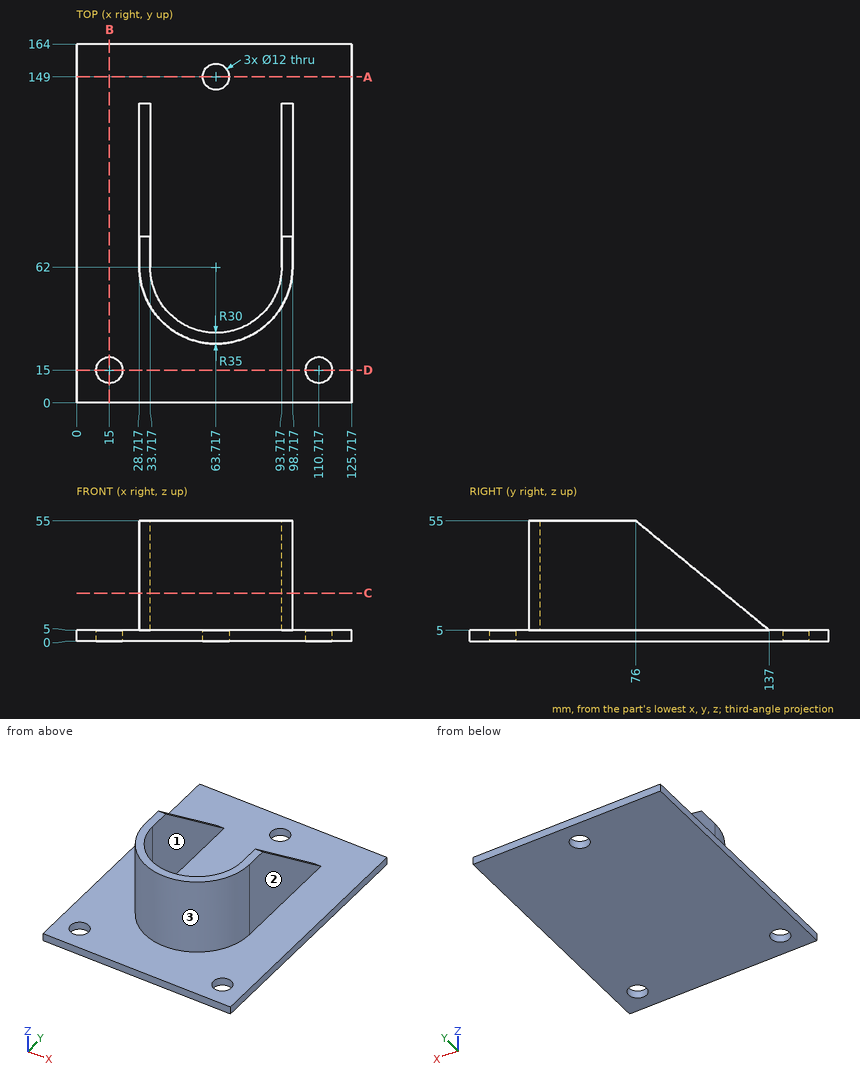
Input: dimensioned drawing with shaded views. Units: mm. Origin: part minimum x, y, z. Round coordinates to 2 decimals unless told otherwise and drop trailing zeros. Order: outer loops, then holes, each group sorted by start corner. A loop starts at its lowest first (then second) coordinate and runs counter-clockwise, first axis right, second up. Notation, with made-up numbers: (-23.75, 67) -> (13.25, 67) arc R24 ccw to (13.25, 84) -> close; hole circle Ø7 at (82, -20.5). An arc over 180 degrees is marked (long way). One line per item, written item: value. Start each with the question number.
Q1. Section query C-C (z = 22). Return the cut outline in (x, y), plus the area to 3 significant figures.
Q2. Section query D-D (y = 15). Return the cut outline in (x, z).
Q3. Section query B-B (x = 15). Return the cut outline in (y, z).
Q4. Draft query along X for the marked faces 1, 2 and 3. Return one class per face: pulls with the +X half, pulls with the -X half, needs draft (parallel to the pull), parting line crosses it, or undercut.
Q5. Section query A-A (y = 149). Return the cut outline in (x, z).
Q6. Pin query (flat end, axial travel): pin 1 (25 mm diameter, centred on y = 105, z = 39.5, fed in from -X); pin 2 (10 mm diameter, centred on y = 45, z = 11.5, fed in from +X); pin 3 (5 mm diameter, centred on y = 91.5, z = 32.5, fed in from +X). Return the tip coordinate at first contact, or that it passes through.
Q7. Material intervals for probe 1 along X at (y, z) = (72, 43); probe 2 along Z at (x, y) = (59.5, 21); probe 3 along Y at (x, z) = (15, 1.6), sorted ascending.
Findings below:
1. outline: (28.72, 62) arc R35 ccw to (98.72, 62) -> (98.72, 116.26) -> (93.72, 116.26) -> (93.72, 62) arc R30 cw to (33.72, 62) -> (33.72, 116.26) -> (28.72, 116.26) -> close
1. area: 1,050 mm²
2. outline: (0, 0) -> (9, 0) -> (9, 5) -> (0, 5) -> close; (21, 0) -> (104.72, 0) -> (104.72, 5) -> (21, 5) -> close; (116.72, 0) -> (125.72, 0) -> (125.72, 5) -> (116.72, 5) -> close
3. outline: (0, 0) -> (9, 0) -> (9, 5) -> (0, 5) -> close; (21, 0) -> (164, 0) -> (164, 5) -> (21, 5) -> close
4. face 1: undercut
4. face 2: pulls with the +X half
4. face 3: parting line crosses it
5. outline: (0, 0) -> (57.72, 0) -> (57.72, 5) -> (0, 5) -> close; (69.72, 0) -> (125.72, 0) -> (125.72, 5) -> (69.72, 5) -> close
6. pin 1: x = 28.72
6. pin 2: x = 96.6
6. pin 3: x = 98.72
7. probe 1: 28.72 to 33.72, 93.72 to 98.72
7. probe 2: 0 to 5
7. probe 3: 0 to 9, 21 to 164
